from build123d import *

# Parameters (mm, degrees)
SKETCH1_W             = 80
SKETCH1_H             = 80
BOSS_EXTRUDE1_DEPTH   = 40
M30_CLEARANCE_HOLE1_D = 35
FILLET1_R             = 5
CHAMFER1_SIZE         = 0.5


with BuildPart() as part:
    # Sketch1 → Boss-Extrude1 (new body)
    with BuildSketch(Plane(origin=(0, 15, 0), x_dir=(1, 0, 0), z_dir=(0, 1, 0))):
        Rectangle(SKETCH1_W, SKETCH1_H)
    extrude(amount=-BOSS_EXTRUDE1_DEPTH)

    # M30 Clearance Hole1 (through all)
    with Locations(Plane(origin=(0, 15, 0), x_dir=(1, 0, 0), z_dir=(0, 1, 0))):
        with Locations((0, 0)):
            Hole(M30_CLEARANCE_HOLE1_D / 2)

    # Fillet1
    fillet1_edges = [part.edges().sort_by_distance(p)[0] for p in [
        (-40, -5, -40),
        (40, -5, -40),
        (40, -5, 40),
        (-40, -5, 40),
    ]]
    fillet(fillet1_edges, radius=FILLET1_R)

    # Chamfer1
    chamfer1_edges = [part.edges().sort_by_distance(p)[0] for p in [
        (0, 15, 40),
        (-40, 15, 0),
        (40, 15, 0),
        (0, 15, -40),
        (-38.535533906, 15, -38.535533906),
        (38.535533906, 15, -38.535533906),
        (-38.535533906, 15, 38.535533906),
        (38.535533906, 15, 38.535533906),
    ]]
    chamfer(chamfer1_edges, length=CHAMFER1_SIZE)


solid = part.part
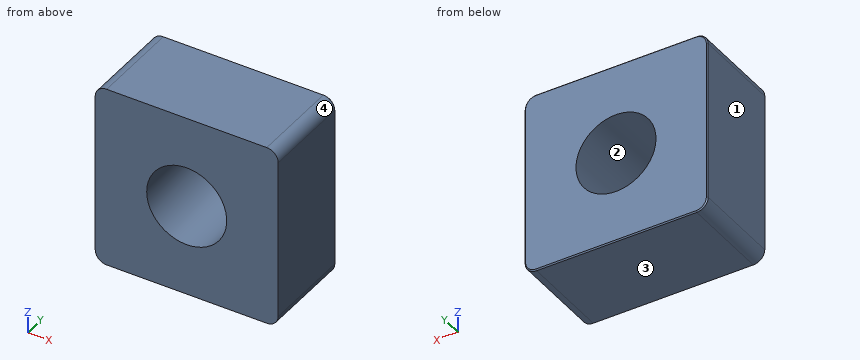
Design review of the part built by this model. Coordinates are the model's own, in mm. Face numbers are marked on the shaded views. Round coordinates to 2 decimals unless told otherwise and drop trailing zeros. Write each loop counter-clockwise with the first axis right and the second up, starting at its lowest first coordinate (ties: lowest second). Pieces come first, ordered by that corner, then holes. Notation, with made-up numbers: (53.5, -2.5) - (111.5, -2.5) arc R17 ccw to (111.5, 7.5) - close; hole circle Ø2 at (3, -4.75). An arc over 180 degrees is marked (long way). Use a Markdown table: item, result. Add a question column.
1. Mouldability with a two-part tool opening along Z and no side actions: class the marked faces 1, 2, 3 and 4 as +Z half, -Z half, draft (parallel to the pull), parting line (faces both ways), or undercut.
2. We need section C-C (z = 0). State the section outline as (x, y) points.
3. Wall thickness on probe 1 along Z at (x, y) = (0, -1.5); probe 2 along X at (y, z) = (-5, 10); probe 3 along X at (y, z) = (11, -12): over which ranges is each line inside the solid? List them lowest first.
4. We need section B-B (y = -6). State the section outline as (x, z) points.
5. We need section A-A (x = 0). State the section outline as (y, z) points.
Output:
| question | item | result |
|---|---|---|
| 1 | face 1 | draft |
| 1 | face 2 | undercut |
| 1 | face 3 | -Z half |
| 1 | face 4 | +Z half |
| 2 | outline | (-40, -25) - (-17.5, -25) - (-17.5, 15) - (-39.5, 15) - (-40, 14.5) - close; (17.5, -25) - (40, -25) - (40, 14.5) - (39.5, 15) - (17.5, 15) - close |
| 3 | probe 1 | z = -40 to -17.5, 17.5 to 40 |
| 3 | probe 2 | x = -40 to -14.36, 14.36 to 40 |
| 3 | probe 3 | x = -40 to -12.74, 12.74 to 40 |
| 4 | outline | (-40, -35) arc R5 ccw to (-35, -40) - (35, -40) arc R5 ccw to (40, -35) - (40, 35) arc R5 ccw to (35, 40) - (-35, 40) arc R5 ccw to (-40, 35) - close; hole circle Ø35 at (0, 0) |
| 5 | outline | (-25, -40) - (14.5, -40) - (15, -39.5) - (15, -17.5) - (-25, -17.5) - close; (-25, 17.5) - (15, 17.5) - (15, 39.5) - (14.5, 40) - (-25, 40) - close |
